from build123d import *

# Parameters (mm, degrees)
EXTRUDE_THIN1_DEPTH = 110
SKETCH2_R           = 15.1
CUT_EXTRUDE1_DEPTH  = 124.389626793


with BuildPart() as part:
    # Sketch1 → Extrude-Thin1 (new body)
    with BuildSketch(Plane.XY):
        with BuildLine():
            Line((-25, 21), (-25, -21))
            ThreePointArc((-25, -21), (-23.828427125, -23.828427125), (-21, -25))
            Line((-21, -25), (21, -25))
            ThreePointArc((21, -25), (23.828427125, -23.828427125), (25, -21))
            Line((25, -21), (25, 21))
            ThreePointArc((25, 21), (23.828427125, 23.828427125), (21, 25))
            Line((21, 25), (-21, 25))
            ThreePointArc((-21, 25), (-23.828427125, 23.828427125), (-25, 21))
        make_face()
        with BuildLine():
            Line((-22, 21), (-22, -21))
            ThreePointArc((-22, -21), (-21.707106781, -21.707106781), (-21, -22))
            Line((-21, -22), (21, -22))
            ThreePointArc((21, -22), (21.707106781, -21.707106781), (22, -21))
            Line((22, -21), (22, 21))
            ThreePointArc((22, 21), (21.707106781, 21.707106781), (21, 22))
            Line((21, 22), (-21, 22))
            ThreePointArc((-21, 22), (-21.707106781, 21.707106781), (-22, 21))
        make_face(mode=Mode.SUBTRACT)
    extrude(amount=EXTRUDE_THIN1_DEPTH)

    # Sketch2 → Cut-Extrude1 (cut, through all)
    with BuildSketch(Plane(origin=(25, 0, 0), x_dir=(0, 0, -1), z_dir=(1, 0, 0))):
        with Locations((-20, 0)):
            Circle(SKETCH2_R)
    extrude(amount=-CUT_EXTRUDE1_DEPTH, mode=Mode.SUBTRACT)


solid = part.part
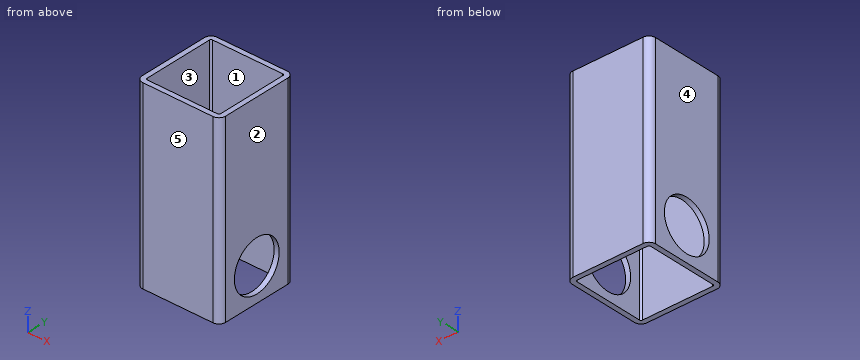
Design review of the part built by this model. Coordinates are the model's own, in mm. Face numbers are marked on the shaded views. A direction names the side the tool comes from. Coordinates: 2 decimals unless noted, no trailing zeros. Loops run counter-clockwise (first coordinate to the right, second up) from the corner with the lowest first, then second, coordinate; pieces in that order, holes last. Notation, with made-up numbers: M -27.75,32 L 21.25,32 A7 cw 21.25,44 Z; hole C 33.5,51 d10. An arc over 180 degrees is marked long. Answer as CSV lines item,"result".
Item 1: Add section B-B on z = 99.5. State the section outline as (x, y) points, plus the area to 3 significant figures.
Answer list:
outline,"M -25,-21 A4 ccw -21,-25 L 21,-25 A4 ccw 25,-21 L 25,21 A4 ccw 21,25 L -21,25 A4 ccw -25,21 Z; hole M -22,-21 A1 ccw -21,-22 L 21,-22 A1 ccw 22,-21 L 22,21 A1 ccw 21,22 L -21,22 A1 ccw -22,21 Z"
area,"551 mm²"
Item 2: For P1, Ø24, axis at y = 0, z = 20, coming from the +X side, flat-tipped, find the tip position at first contact; note if it passes through.
Answer list:
P1,"through"
Item 3: Add section C-C on x = -18. State the section outline as (y, z) points, plus the area to 3 significant figures.
Answer list:
outline,"M -25,0 L -22,0 L -22,110 L -25,110 Z; M 22,0 L 25,0 L 25,110 L 22,110 Z"
area,"660 mm²"
Item 4: The part is to be moulded in two halves that separate along Y. For the marked faces 3, 4 and 5, say which applies: pulls with the +Y half, pulls with the -Y half, needs draft (parallel to the pull), parting line crosses it, or undercut.
Answer list:
face 3,"undercut"
face 4,"needs draft"
face 5,"pulls with the -Y half"
Item 5: For probe 1 along X at (y, z) = (14, 36); probe 2 along Y at (x, z) = (22.95, 20), list the stretches that pass through material, from the lowest coordinate up.
Answer list:
probe 1,"-25 to -22, 22 to 25"
probe 2,"-24.49 to -15.1, 15.1 to 24.49"
Item 6: Add section A-A on y = 0. State the section outline as (x, z) points, plus the area to 3 significant figures.
Answer list:
outline,"M -25,0 L -22,0 L -22,4.9 L -25,4.9 Z; M -25,35.1 L -22,35.1 L -22,110 L -25,110 Z; M 22,0 L 25,0 L 25,4.9 L 22,4.9 Z; M 22,35.1 L 25,35.1 L 25,110 L 22,110 Z"
area,"479 mm²"
Item 7: Machinability: for the marked faces 1 and 2, which of the approach directions +Z, -Z, +X, -X, +Y, -Y give a long, thin tool a straight path to every point of the face, cutting with its end or side? Answer none if there is none.
Answer list:
face 1,"+Z, -Z"
face 2,"+Z, -Z, +X, +Y, -Y"
Item 8: Add section D-D on z = 20. State the section outline as (x, y) points.
Answer list:
outline,"M -25,-21 A4 ccw -21,-25 L 21,-25 A4 ccw 25,-21 L 25,-15.1 L 22,-15.1 L 22,-21 A1 cw 21,-22 L -21,-22 A1 cw -22,-21 L -22,-15.1 L -25,-15.1 Z; M -25,15.1 L -22,15.1 L -22,21 A1 cw -21,22 L 21,22 A1 cw 22,21 L 22,15.1 L 25,15.1 L 25,21 A4 ccw 21,25 L -21,25 A4 ccw -25,21 Z"
